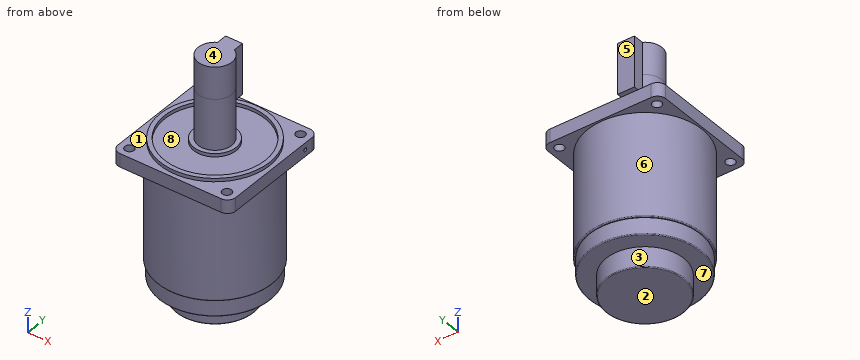
from build123d import *

# Parameters (mm, degrees)
SKETCH_3_W                  = 70
SKETCH_3_H                  = 70
EXTRUDE_1_DEPTH             = 8
SKETCH_5_W                  = 32
SKETCH_5_H                  = 4
SKETCH_5_W_2                = 2
SKETCH_5_H_2                = 2.6
SKETCH_4_R                  = 2.75
CUT_EXTRUDE_1_DEPTH         = 8
PATTERN_CIRCULAR_1_COUNT    = 4
FILLET_1_R                  = 4.9
SKETCH_7_R                  = 1.12
CUT_EXTRUDE_2_DEPTH         = 1
CUT_EXTRUDE_START           = -25
CUT_EXTRUDE_7_DEPTH         = 25
CHAMFER_2_SIZE              = 0.38
SKETCH_35_R                 = 6
EXTRUDE_7_DEPTH             = 4
FILLET_4_R                  = 0.5
SCALE_1_SCALE               = 0.5
EXTRUDE_8_REACH             = 68.293
SKETCH_37_R                 = 5
EXTRUDE_8_DIRECTION_2_DEPTH = 9.5
SKETCH_38_W                 = 5
SKETCH_38_H                 = 5
EXTRUDE_9_DEPTH             = 15


with BuildPart() as part:
    # 草图3 → 凸台-拉伸1 (new body)
    with BuildSketch(Plane.XY):
        Rectangle(SKETCH_3_W, SKETCH_3_H)
    extrude(amount=-EXTRUDE_1_DEPTH)

    # 草图5 → 旋转1 (revolve)
    with BuildSketch(Plane(origin=(0, 0, 0), x_dir=(0, 0, -1), z_dir=(1, 0, 0)), mode=Mode.PRIVATE) as revolve_1_sk:
        with Locations((-16, 2)):
            Rectangle(SKETCH_5_W, SKETCH_5_H)
        with Locations((-1, 31.2)):
            Rectangle(SKETCH_5_W_2, SKETCH_5_H_2)
        with Locations((-1, 11.3)):
            Rectangle(SKETCH_5_W_2, SKETCH_5_H_2)
    revolve(revolve_1_sk.sketch.rotate(Axis((0, 0, 32), (0, 0, -1)), 90), axis=Axis((0, 0, 32), (0, 0, -1)))

    # 草图4 → 切除-拉伸1 (cut)
    with BuildSketch(Plane.XY):
        with Locations((28.991378029, 28.991378029)):
            Circle(SKETCH_4_R)
    cut_extrude_1 = extrude(amount=-CUT_EXTRUDE_1_DEPTH, mode=Mode.SUBTRACT)

    # 阵列(圆周)1: 切除-拉伸1 ×4 about axis
    pattern_circular_1_axis = Axis((0, 0, 0), (0, 0, 1))
    for i in range(1, PATTERN_CIRCULAR_1_COUNT):
        add(cut_extrude_1.rotate(pattern_circular_1_axis, i * 360 / PATTERN_CIRCULAR_1_COUNT), mode=Mode.SUBTRACT)

    # 圆角1
    fillet_1_edges = [part.edges().sort_by_distance(p)[0] for p in [
        (-35, 35, -4),
        (35, 35, -4),
        (35, -35, -4),
        (-35, -35, -4),
    ]]
    fillet(fillet_1_edges, radius=FILLET_1_R)

    # 草图7 → 切除-拉伸2 (cut)
    with BuildSketch(Plane(origin=(35, 0, 0), x_dir=(0, 0, -1), z_dir=(1, 0, 0))):
        with Locations((4, 24.7)):
            Circle(SKETCH_7_R)
    extrude(amount=-CUT_EXTRUDE_2_DEPTH, mode=Mode.SUBTRACT)

    # 草图31 → 切除-拉伸7 (cut)
    with BuildSketch(Plane.XY.offset(32).offset(CUT_EXTRUDE_START)):
        with BuildLine():
            Line((3.5, 1.936491673), (3.5, -1.936491673))
            ThreePointArc((3.5, -1.936491673), (4, 0), (3.5, 1.936491673))
        make_face()
    extrude(amount=CUT_EXTRUDE_7_DEPTH, mode=Mode.SUBTRACT)

    # 倒角2
    chamfer_2_edges = [part.edges().sort_by_distance(p)[0] for p in [
        (-4, 0, 32),
    ]]
    chamfer(chamfer_2_edges, length=CHAMFER_2_SIZE)

    # 草图35 → 凸台-拉伸7 (add)
    with BuildSketch(Plane.XY):
        Circle(SKETCH_35_R)
    extrude(amount=EXTRUDE_7_DEPTH)

    # 草图8 → 旋转3 (revolve)
    with BuildSketch(Plane(origin=(0, 0, 0), x_dir=(0, 0, -1), z_dir=(1, 0, 0))):
        Polygon((8, 34), (69.2, 34), (69.2, 33), (79, 33), (79, 23), (91, 23), (91, 0), (8, 0), align=None)
    revolve(axis=Axis((0, 0, -91), (0, 0, 1)))

    # 圆角4
    fillet_4_edges = [part.edges().sort_by_distance(p)[0] for p in [
        (0, -34, -69.2),
        (0, -33, -79),
        (0, -23, -91),
    ]]
    fillet(fillet_4_edges, radius=FILLET_4_R)


with BuildPart() as part_1:
    # 缩放比例1: scaled about (-0.000807306, -0.000306882, -40.615231306)
    add(part.part.scale(SCALE_1_SCALE).moved(Location((-0.000403653, -0.000153441, -20.307615653))))

    # 草图37 → 凸台-拉伸8 (add, up to next)
    with BuildSketch(Plane.XY.offset(-4.307615654), mode=Mode.PRIVATE) as extrude_8_sk1:
        with Locations(Location((0, 0, 0), (0, 0, 110.815805109))):
            Circle(SKETCH_37_R)
    extrude_8_tool1 = extrude(extrude_8_sk1.sketch, amount=-EXTRUDE_8_REACH, mode=Mode.PRIVATE) - part_1.part
    add(extrude_8_tool1.solids().sort_by_distance((0, 0, -4.307616))[0])

    # 草图37 → 凸台-拉伸8 direction 2 (add)
    with BuildSketch(Plane.XY.offset(-4.307615654)):
        with Locations(Location((0, 0, 0), (0, 0, 110.815805109))):
            Circle(SKETCH_37_R)
    extrude(amount=EXTRUDE_8_DIRECTION_2_DEPTH)

    # 草图38 → 凸台-拉伸9 (add)
    with BuildSketch(Plane.XY.offset(5.192384346)):
        with Locations((0, 5)):
            Rectangle(SKETCH_38_W, SKETCH_38_H)
    extrude(amount=-EXTRUDE_9_DEPTH)


solid = part_1.part
Check sheet for the modelled part. Datum: model origin and axes. Units: mm. Face numbers are marked on the shaded views. A direction names the side the tool comes from. Round coordinates to 2 decimals unless told otherwise and drop trailing zeros. Order: outer loops, then holes, each group sorted by start corner. A loop starts at its lowest first (then second) coordinate and runs counter-clockwise, first axis right, second up.
(1) Cross-section at A-A, the plane z = -3. Enter the section's corners in (x, y), and give its area (3 significant figures).
(2) Access from +Z, -Z, +X, -X, +Y, -Y to the whole of each face (thin tool, end or side, straight path). Record for the marked faces 1, 2, 3, 4 and 5.
(3) Scan lines: probe 1 along Y at (x, z) = (-15, -20.5); probe 2 along Z at (x, y) = (14.5, -9); probe 3 along Z at (x, y) = (13.5, -7.5). Record each from-to range of solid material in increasing order.
(4) Go/stop test with flat-tipped pins: P1, Ø8, axis at x = -12.5, z = -58, coming from the +Y side; P2, Ø4.5, axis at x = 14.5, y = 14.5, coming from the +Z side; P3, Ø5.5, axis at x = -1, z = -1, coming from the +Y side. Record where each tip stops, or that it passes through.
(5) Draft check along Y on the marked faces 6, 7 and 8. Enter one of: pulls with the +Y half, pulls with the -Y half, needs draft (parallel to the pull), parting line crosses it, or undercut.
(6) Cross-section at B-B, the plane z = -25.5. Enter the section's corners in (x, y), and give its area (3 significant figures).
Check sheet entries:
1. outline: (-2.5, 4.33) arc R5 ccw (long way) to (2.5, 4.33) - (2.5, 7.5) - (-2.5, 7.5) - close
1. area: 92.1 mm2
2. face 1: +Z
2. face 2: -Z, +X, -X, +Y, -Y
2. face 3: -Z
2. face 4: +Z, +X, -X, +Y, -Y
2. face 5: +Z, +X, -X, +Y
3. probe 1: y = -17.5 to -15.78, -13.22 to 13.22, 15.77 to 17.5
3. probe 2: z = -24.31 to -20.31
3. probe 3: z = -59.81 to -19.31
4. P1: stops at y = 14.14
4. P2: stops at z = -20.31
4. P3: stops at y = 7.5
5. face 6: parting line crosses it
5. face 7: needs draft
5. face 8: undercut
6. outline: circle Ø34 at (0, 0)
6. area: 908 mm2
